Input: part model. Units: mm. Frame: model coordinates. A direction names the side the tool comes from. Coordinates: 2 decimals unless noted, no trailing zeros. Loops run counter-clockwise (first coordinate to the right, second up) from the corner with the lowest first, then second, coordinate; pieces in that order, holes last. Notation, with made-up numbers: (-19, 37) -> (-12, 37) arc R10 cw to (-12, 42) -> close; hole circle Ø6 at (-19.5, -30). An arc over 180 degrees is marked (long way). Put each result on its own line as item: value. Start each with the question number.
1) Set-up query: faces 1 (the cylindrical face through (19.394, 99.972, 12.365)), 2 (the conical face through (-5.295, 80.596, 23.843)), 3 (the cylindrical face through (0.2, 92.9, 32.5)). Return all of +Z, -Z, +X, -X, +Y, -Y with unobstructed straight access to the full face (end or side cutting, diameter ignored); none if empty.
2) Contact query for flat-ended pins moving along their axis: P1, Ø1.5, axis at y = 44, z = 0.5, coming from the +X side; P2, Ø12, axis at x = 3.5, z = -37.5, coming from the -Y side; P3, Ø11, axis at x = 50, z = 0, coming from the +Y side; P4, Ø3, axis at y = 20.5, z = 6.5, coming from the -X side. Output: stop coordinate, or through.
3) Pull-direction query (Z, two-part tool) for faces 4 (the cylindrical face through (43.902, 7.098, 41.763)), 5 (the cylindrical face through (-23.122, 26.114, -30.156)), 6 (the flat face through (22, 0, -24)), 7 (the flat face through (-34.07, 92.93, 19.77)); classes: pulls with the +Z half, pulls with the -Z half, needs draft (parallel to the pull), parting line crosses it, or undercut.
4) Material intervals for L1, parallel to X at y = 11.25, z = -38; L2, parallel to Y at x = -40, z = 4; L3, parallel to Z at x = 2.5, y = 35, sorted ascending.
5) Cut plane A-A (y = 91). Return the cut outline in (x, z) (3 decimals).
6) Cut plane B-B (z = 2.5). State how many separate pieces and enclosed holes the cut face has, plus the area to 3 significant figures.
7) Cut plane C-C (y = 71.5). Return the cut outline in (x, z).
from build123d import *

# Parameters (mm, degrees)
BASE_FLANGE_DEPTH               = 14
BASE_BOSS_SKETCH_R              = 38
BASE_BOSS_76_DEPTH              = 22
NECK_LOFT_UPPER_PROFILE_46_R    = 23
NECK_LOFT_LOWER_PROFILE_R       = 28
TOP_FLANGE_DEPTH                = 10
TOP_SPIGOT_SKETCH_R             = 23
TOP_SPIGOT_46_DEPTH             = 4
BOTTOM_BORE_SKETCH_R            = 30
BOTTOM_BORE_60_DEPTH            = 104.831594421
BASE_MOUNTING_HOLES_SKETCH_R    = 7
BASE_MOUNTING_HOLES_4X_14_DEPTH = 120.033608699
TOP_FLANGE_HOLES_2X_12_REACH    = 128.606
TOP_FLANGE_HOLES_SKETCH_R       = 6
BASE_BOSS_FILLET_R2_5_R         = 2.5


with BuildPart() as part:
    # Base Flange Sketch → Base Flange (new body)
    with BuildSketch(Plane(origin=(0, 0, 0), x_dir=(1, 0, 0), z_dir=(0, 1, 0))):
        with BuildLine():
            ThreePointArc((-32.088888889, 50.690893012), (-47.899494937, 47.899494937), (-50.690893012, 32.088888889))
            ThreePointArc((-50.690893012, 32.088888889), (-43.584312217, 0), (-50.690893012, -32.088888889))
            ThreePointArc((-50.690893012, -32.088888889), (-47.899494937, -47.899494937), (-32.088888889, -50.690893012))
            ThreePointArc((-32.088888889, -50.690893012), (0, -43.584312217), (32.088888889, -50.690893012))
            ThreePointArc((32.088888889, -50.690893012), (47.899494937, -47.899494937), (50.690893012, -32.088888889))
            ThreePointArc((50.690893012, -32.088888889), (43.584312217, 0), (50.690893012, 32.088888889))
            ThreePointArc((50.690893012, 32.088888889), (47.899494937, 47.899494937), (32.088888889, 50.690893012))
            ThreePointArc((32.088888889, 50.690893012), (0, 43.584312217), (-32.088888889, 50.690893012))
        make_face()
    extrude(amount=BASE_FLANGE_DEPTH)

    # Base Boss Sketch → Base Boss Ø76 (add)
    with BuildSketch(Plane(origin=(0, 14, 0), x_dir=(1, 0, 0), z_dir=(0, 1, 0))):
        with Locations(Location((0, 0, 0), (0, 0, 270))):
            Circle(BASE_BOSS_SKETCH_R)
    extrude(amount=BASE_BOSS_76_DEPTH)

    # Ball Body Profile → Ball Body (revolve)
    with BuildSketch(Plane(origin=(0, 0, 0), x_dir=(0, 0, -1), z_dir=(1, 0, 0)), mode=Mode.PRIVATE) as ball_body_sk:
        with BuildLine():
            Line((0, 62), (-28, 62))
            ThreePointArc((-28, 62), (-35.468382669, 49.94937795), (-38, 36))
            Line((-38, 36), (0, 36))
            Line((0, 36), (0, 62))
        make_face()
    revolve(ball_body_sk.sketch.rotate(Axis((0, 14, 0), (0, 1, 0)), 180), axis=Axis((0, 14, 0), (0, 1, 0)))

    # Neck Loft Upper Profile Ø46 → Neck Loft section 0
    with BuildSketch(Plane(origin=(0, 88, 0), x_dir=(1, 0, 0), z_dir=(0, 1, 0))):
        Circle(NECK_LOFT_UPPER_PROFILE_46_R)
    # Neck Loft Lower Profile → Neck Loft section 1
    with BuildSketch(Plane(origin=(0, 62, 0), x_dir=(1, 0, 0), z_dir=(0, 1, 0))):
        Circle(NECK_LOFT_LOWER_PROFILE_R)
    loft()

    # Top Flange Sketch → Top Flange (add)
    with BuildSketch(Plane(origin=(0, 88, 0), x_dir=(1, 0, 0), z_dir=(0, 1, 0))):
        with BuildLine():
            Line((-54.73, 9.931117762), (-13.975, 29.341938842))
            ThreePointArc((-13.975, 29.341938842), (0, 32.5), (13.975, 29.341938842))
            Line((13.975, 29.341938842), (54.73, 9.931117762))
            ThreePointArc((54.73, 9.931117762), (61, 0), (54.73, -9.931117762))
            Line((54.73, -9.931117762), (13.975, -29.341938842))
            ThreePointArc((13.975, -29.341938842), (0, -32.5), (-13.975, -29.341938842))
            Line((-13.975, -29.341938842), (-54.73, -9.931117762))
            ThreePointArc((-54.73, -9.931117762), (-61, 0), (-54.73, 9.931117762))
        make_face()
    extrude(amount=TOP_FLANGE_DEPTH)

    # Top Spigot Sketch → Top Spigot Ø46 (add)
    with BuildSketch(Plane(origin=(0, 98, 0), x_dir=(1, 0, 0), z_dir=(0, 1, 0))):
        with Locations(Location((0, 0, 0), (0, 0, 270))):
            Circle(TOP_SPIGOT_SKETCH_R)
    extrude(amount=TOP_SPIGOT_46_DEPTH)

    # Ball Groove Profile → Ball Groove (revolve, cut)
    with BuildSketch(Plane.XY, mode=Mode.PRIVATE) as ball_groove_sk:
        Polygon((0, 102), (14, 102), (22.94149422, 56), (0, 56), align=None)
    revolve(ball_groove_sk.sketch.rotate(Axis((0, 102, 0), (0, -1, 0)), 90), axis=Axis((0, 102, 0), (0, -1, 0)), mode=Mode.SUBTRACT)

    # Inner Cavity Profile → Inner Cavity (revolve, cut)
    with BuildSketch(Plane.XY, mode=Mode.PRIVATE) as inner_cavity_sk:
        with BuildLine():
            Line((0, 36), (30, 36))
            ThreePointArc((30, 36), (28.297120073, 46.644573206), (22.94149422, 56))
            Line((22.94149422, 56), (0, 56))
            Line((0, 56), (0, 36))
        make_face()
    revolve(inner_cavity_sk.sketch.rotate(Axis((0, 56, 0), (0, -1, 0)), 90), axis=Axis((0, 56, 0), (0, -1, 0)), mode=Mode.SUBTRACT)

    # Bottom Bore Sketch → Bottom Bore Ø60 (cut, through all)
    with BuildSketch(Plane(origin=(0, 36, 0), x_dir=(1, 0, 0), z_dir=(0, 1, 0))):
        with Locations(Location((0, 0, 0), (0, 0, 270))):
            Circle(BOTTOM_BORE_SKETCH_R)
    extrude(amount=-BOTTOM_BORE_60_DEPTH, mode=Mode.SUBTRACT)

    # Base Mounting Holes Sketch → Base Mounting Holes 4xØ14 (cut, through all)
    with BuildSketch(Plane(origin=(0, 14, 0), x_dir=(1, 0, 0), z_dir=(0, 1, 0))):
        with Locations(Location((38, 38, 0), (0, 0, 270))):
            Circle(BASE_MOUNTING_HOLES_SKETCH_R)
        with Locations(Location((38, -38, 0), (0, 0, 270))):
            Circle(BASE_MOUNTING_HOLES_SKETCH_R)
        with Locations(Location((-38, 38, 0), (0, 0, 270))):
            Circle(BASE_MOUNTING_HOLES_SKETCH_R)
        with Locations(Location((-38, -38, 0), (0, 0, 270))):
            Circle(BASE_MOUNTING_HOLES_SKETCH_R)
    extrude(amount=-BASE_MOUNTING_HOLES_4X_14_DEPTH, mode=Mode.SUBTRACT)

    # Top Flange Holes Sketch → Top Flange Holes 2xØ12 (cut, up to next)
    with BuildSketch(Plane(origin=(0, 98, 0), x_dir=(1, 0, 0), z_dir=(0, 1, 0)), mode=Mode.PRIVATE) as top_flange_holes_2x_12_sk1:
        with Locations(Location((50, 0, 0), (0, 0, 270))):
            Circle(TOP_FLANGE_HOLES_SKETCH_R)
    top_flange_holes_2x_12_tool1 = extrude(top_flange_holes_2x_12_sk1.sketch, amount=-TOP_FLANGE_HOLES_2X_12_REACH, mode=Mode.PRIVATE) & part.part
    # Top Flange Holes Sketch → Top Flange Holes 2xØ12 (cut, up to next)
    with BuildSketch(Plane(origin=(0, 98, 0), x_dir=(1, 0, 0), z_dir=(0, 1, 0)), mode=Mode.PRIVATE) as top_flange_holes_2x_12_sk2:
        with Locations(Location((-50, 0, 0), (0, 0, 270))):
            Circle(TOP_FLANGE_HOLES_SKETCH_R)
    top_flange_holes_2x_12_tool2 = extrude(top_flange_holes_2x_12_sk2.sketch, amount=-TOP_FLANGE_HOLES_2X_12_REACH, mode=Mode.PRIVATE) & part.part
    add(top_flange_holes_2x_12_tool1.solids().sort_by_distance((50, 98, 0))[0], mode=Mode.SUBTRACT)
    add(top_flange_holes_2x_12_tool2.solids().sort_by_distance((-50, 98, 0))[0], mode=Mode.SUBTRACT)

    # Base Boss Fillet R2.5
    base_boss_fillet_r2_5_edges = [part.edges().sort_by_distance(p)[0] for p in [
        (0, 14, 43.584312217),
        (47.899494937, 14, 47.899494937),
        (43.584312217, 14, 0),
        (47.899494937, 14, -47.899494937),
        (0, 14, -38),
        (0, 14, -43.584312217),
        (-47.899494937, 14, -47.899494937),
        (-43.584312217, 14, 0),
        (-47.899494937, 14, 47.899494937),
    ]]
    fillet(base_boss_fillet_r2_5_edges, radius=BASE_BOSS_FILLET_R2_5_R)


solid = part.part
Results found:
1. face 1: +Y
1. face 2: none
1. face 3: +Z, +Y
2. P1: stops at x = 37.36
2. P2: stops at y = 0
2. P3: passes through
2. P4: stops at x = -37.67
3. face 4: undercut
3. face 5: parting line crosses it
3. face 6: needs draft
3. face 7: pulls with the +Z half
4. L1: x = -52 to -45, -31 to 31, 45 to 52
4. L2: y = 0 to 14.02, 88 to 98
4. L3: z = -37.92 to -29.9, 29.9 to 37.92
5. outline: (-54.73, -9.931) -> (-13.975, -29.342) arc R32.5 ccw to (13.975, -29.342) -> (54.73, -9.931) arc R11 ccw to (54.73, 9.931) -> (13.975, 29.342) arc R32.5 ccw to (-13.975, 29.342) -> (-54.73, 9.931) arc R11 ccw to start; hole circle Ø12 at (-50, 0); hole circle Ø32.276 at (0, 0); hole circle Ø12 at (50, 0)
6. separate pieces: 4
6. enclosed holes: 0
6. area: 2,250 mm2
7. outline: circle Ø52.35 at (0, 0); hole circle Ø39.86 at (0, 0)
